```python
from build123d import *

# Parameters (mm, degrees)
BOSS_EXTRUDE1_DEPTH = 50
CUT_EXTRUDE1_DEPTH  = 30
CUT_EXTRUDE2_REACH  = 359.071
SKETCH3_R           = 25


with BuildPart() as part:
    # Sketch1 → Boss-Extrude1 (new body)
    with BuildSketch(Plane(origin=(0, 0, 0), x_dir=(1, 0, 0), z_dir=(0, 1, 0))):
        with BuildLine():
            Line((-220, -250), (220, -250))
            ThreePointArc((220, -250), (241.213203436, -241.213203436), (250, -220))
            Line((250, -220), (250, 220))
            ThreePointArc((250, 220), (241.213203436, 241.213203436), (220, 250))
            Line((220, 250), (-220, 250))
            ThreePointArc((-220, 250), (-241.213203436, 241.213203436), (-250, 220))
            Line((-250, 220), (-250, -220))
            ThreePointArc((-250, -220), (-241.213203436, -241.213203436), (-220, -250))
        make_face()
    extrude(amount=BOSS_EXTRUDE1_DEPTH)

    # Sketch2 → Cut-Extrude1 (cut)
    with BuildSketch(Plane(origin=(0, 50, 0), x_dir=(1, 0, 0), z_dir=(0, 1, 0))):
        with BuildLine():
            Line((-175, -210), (175, -210))
            ThreePointArc((175, -210), (185.251262658, -185.251262658), (210, -175))
            Line((210, -175), (210, 175))
            ThreePointArc((210, 175), (185.251262658, 185.251262658), (175, 210))
            Line((175, 210), (-175, 210))
            ThreePointArc((-175, 210), (-185.251262658, 185.251262658), (-210, 175))
            Line((-210, 175), (-210, -175))
            ThreePointArc((-210, -175), (-185.251262658, -185.251262658), (-175, -210))
        make_face()
    extrude(amount=-CUT_EXTRUDE1_DEPTH, mode=Mode.SUBTRACT)

    # Sketch3 → Cut-Extrude2 (cut, up to next)
    with BuildSketch(Plane(origin=(0, 50, 0), x_dir=(1, 0, 0), z_dir=(0, 1, 0)), mode=Mode.PRIVATE) as cut_extrude2_sk1:
        with Locations(Location((-210, 210, 0), (0, 0, 270))):
            Circle(SKETCH3_R)
    cut_extrude2_tool1 = extrude(cut_extrude2_sk1.sketch, amount=-CUT_EXTRUDE2_REACH, mode=Mode.PRIVATE) & part.part
    # Sketch3 → Cut-Extrude2 (cut, up to next)
    with BuildSketch(Plane(origin=(0, 50, 0), x_dir=(1, 0, 0), z_dir=(0, 1, 0)), mode=Mode.PRIVATE) as cut_extrude2_sk2:
        with Locations(Location((210, 210, 0), (0, 0, 90))):
            Circle(SKETCH3_R)
    cut_extrude2_tool2 = extrude(cut_extrude2_sk2.sketch, amount=-CUT_EXTRUDE2_REACH, mode=Mode.PRIVATE) & part.part
    # Sketch3 → Cut-Extrude2 (cut, up to next)
    with BuildSketch(Plane(origin=(0, 50, 0), x_dir=(1, 0, 0), z_dir=(0, 1, 0)), mode=Mode.PRIVATE) as cut_extrude2_sk3:
        with Locations(Location((210, -210, 0), (0, 0, 270))):
            Circle(SKETCH3_R)
    cut_extrude2_tool3 = extrude(cut_extrude2_sk3.sketch, amount=-CUT_EXTRUDE2_REACH, mode=Mode.PRIVATE) & part.part
    # Sketch3 → Cut-Extrude2 (cut, up to next)
    with BuildSketch(Plane(origin=(0, 50, 0), x_dir=(1, 0, 0), z_dir=(0, 1, 0)), mode=Mode.PRIVATE) as cut_extrude2_sk4:
        with Locations(Location((-210, -210, 0), (0, 0, 90))):
            Circle(SKETCH3_R)
    cut_extrude2_tool4 = extrude(cut_extrude2_sk4.sketch, amount=-CUT_EXTRUDE2_REACH, mode=Mode.PRIVATE) & part.part
    add(cut_extrude2_tool1.solids().sort_by_distance((-210, 50, -210))[0], mode=Mode.SUBTRACT)
    add(cut_extrude2_tool2.solids().sort_by_distance((210, 50, -210))[0], mode=Mode.SUBTRACT)
    add(cut_extrude2_tool3.solids().sort_by_distance((210, 50, 210))[0], mode=Mode.SUBTRACT)
    add(cut_extrude2_tool4.solids().sort_by_distance((-210, 50, 210))[0], mode=Mode.SUBTRACT)


solid = part.part
```
Geometry check sheet. Reference: the model listing, model coordinates, mm. A direction names the side the tool comes from. Coordinates: 2 decimals unless noted, no trailing zeros. Order: outer loops, then holes, each group sorted by start corner. A loop starts at its lowest first (then second) coordinate and runs counter-clockwise, first axis right, second up.
Q1. Sectioned sample at B-B on z = -82.5. Record the cut outline in (x, y), and give its area (3 significant figures).
Reply:
outline: (-250, 0) - (250, 0) - (250, 50) - (210, 50) - (210, 20) - (-210, 20) - (-210, 50) - (-250, 50) - close
area: 12,400 mm2
Q2. Draft check along X on faces 1 (the face through (-184.981, 35.21, -185.525)), 2 (the face through (3, 25, -250)), 3 (the face through (250, 25, 3)). Enter one of: released by +X, released by -X, zero draft, split by the parting line, or undercut.
Reply:
face 1: undercut
face 2: zero draft
face 3: released by +X
Q3. Sectioned sample at C-C on x = -131. Record the cut outline in (y, z), and give its area (3 significant figures).
Reply:
outline: (0, -250) - (50, -250) - (50, -210) - (20, -210) - (20, 210) - (50, 210) - (50, 250) - (0, 250) - close
area: 12,400 mm2
Q4. Thickness scan on probe 1 along X at (y, z) = (17, -210); probe 2 along Z at (x, y) = (-95.5, 32); probe 3 along X at (y, z) = (4.5, -196.5). Record the ranges inside material, lowest first.
Reply:
probe 1: x = -250 to -235, -185 to 185, 235 to 250
probe 2: z = -250 to -210, 210 to 250
probe 3: x = -250 to -231.04, -188.96 to 188.96, 231.04 to 250
Q5. Tool access check on faces 4 (the face through (185.525, 35.21, -184.981)), 5 (the face through (-240.979, 24.65, -241.445)). Record the directions out of +Z, -Z, +X, -X, +Y, -Y that give a thin tool (end or side, any length) a straight path to the whole face; none if there is none.
Reply:
face 4: +Y
face 5: -Z, -X, +Y, -Y
Q6. Depth check by flat-ended pin: pin 1 Ø3 at (x, z) = (99, 129) entering from +Y. Enter the tip coordinate at first touch or a pass-through.
Reply:
pin 1: stops at y = 20
Q7. Sectioned sample at A-A on y = 14. Record the cut outline in (x, z), and give its area (3 significant figures).
Reply:
outline: (-250, -220) arc R30 ccw to (-220, -250) - (220, -250) arc R30 ccw to (250, -220) - (250, 220) arc R30 ccw to (220, 250) - (-220, 250) arc R30 ccw to (-250, 220) - close; hole circle Ø50 at (-210, -210); hole circle Ø50 at (-210, 210); hole circle Ø50 at (210, -210); hole circle Ø50 at (210, 210)
area: 241,000 mm2
